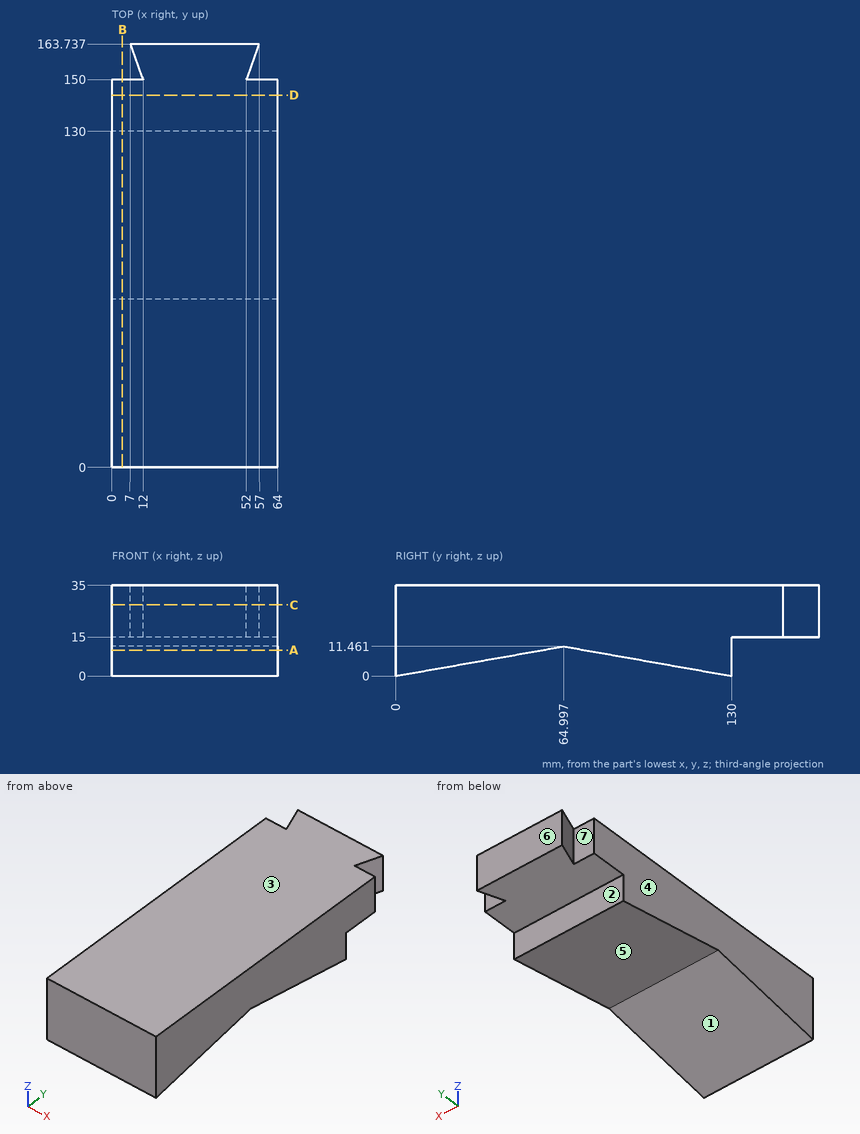
Geometry: see drawing. Coordinates: mm, zero at the bounding-box minimum. A direction names the side the tool comes from. Give positions to 0.01 mm unless a question says otherwise; leave off trailing zeros. Order: outer loops, then holes, each group sorted by start corner. A loop starts at its lowest first (then second) coordinate and runs counter-clockwise, first axis right, second up.
Q1. Ray query, probe 1 along Z at (x, y) = (38.5, 148); probe 2 along Y at (x, z) = (53, 12); probe 3 along Y at (x, z) = (59, 17). Return the intervals inside material, ascending.
Checked values:
probe 1: z = 15 to 35
probe 2: y = 0 to 130
probe 3: y = 0 to 150
Q2. Section A-A on z = 10. Output: boundary loops of the cut face in (x, y) (1 decimal), and give its area (3 significant figures).
Checked values:
outline: (0, 0) - (64, 0) - (64, 56.7) - (0, 56.7) - close; (0, 73.3) - (64, 73.3) - (64, 130) - (0, 130) - close
area: 7,260 mm2
Q3. Section D-D on y = 144. Output: boundary loops of the cut face in (x, z).
Checked values:
outline: (0, 15) - (64, 15) - (64, 35) - (0, 35) - close
Q4. Section C-C on z = 27.5. Output: boundary loops of the cut face in (x, y).
Checked values:
outline: (0, 0) - (64, 0) - (64, 150) - (52, 150) - (57, 163.74) - (7, 163.74) - (12, 150) - (0, 150) - close
Q5. Set-up query: the marked faces 1, 2 and 3. Return all of +Z, -Z, +X, -X, +Y, -Y with unobstructed straight access to the full face (end or side cutting, diameter ignored); none if empty.
Checked values:
face 1: -Z, +X, -X
face 2: -Z, +X, -X, +Y
face 3: +Z, +X, -X, +Y, -Y
Q6. Section B-B on x = 4. Output: boundary loops of the cut face in (y, z), and give its area (4 significant figures).
Checked values:
outline: (0, 0) - (65, 11.46) - (130, 0) - (130, 15) - (150, 15) - (150, 35) - (0, 35) - close
area: 4,205 mm2
Q7. Draft query along Y for the marked faces 4, 5, 6 and 7. Return one class per face: +Y half, -Y half, draft (parallel to the pull), parting line (faces both ways), or undercut.
Checked values:
face 4: draft
face 5: undercut
face 6: +Y half
face 7: undercut
Q8. Contact query for flat-ended pins moving along their axis: pin 1 Ø6 at (x, z) = (61, 20.5) entering from +Y; pin 2 Ø4 at (x, y) = (43, 95) entering from -Z. Output: stop coordinate, or through.
Checked values:
pin 1: stops at y = 150
pin 2: stops at z = 5.82
